Design review of the part built by this model. Coordinates are the model's own, in mm. Face numbers are marked on the shaded views. A direction names the side the tool comes from. Coordinates: 2 decimals unless noted, no trailing zeros. Loops run counter-clockwise (first coordinate to the right, second up) from the corner with the lowest first, then second, coordinate; pieces in that order, holes last. Notation, with made-up numbers: (-12.75, 80.5) -> (42.25, 80.5) arc R18 cw to (42.25, 100.5) -> close; hole circle Ø3 at (-31, 74.25). An arc over 180 degrees is marked (long way). Answer as a JSON object with one key per item and string values.
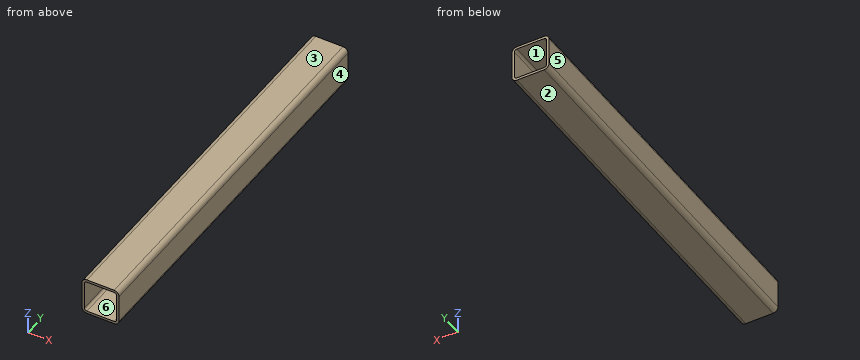
```python
from build123d import *

# Parameters (mm, degrees)
GB_T_6728_2002_SQUARE_HOLLOW_SECTION_60_DEPTH = 620


with BuildPart() as part:
    # Sketch1 → GB/T 6728-2002 square hollow section 60×60×4(1) (new body)
    with BuildSketch(Plane(origin=(0, 0, 0), x_dir=(-1, 0, 0), z_dir=(0, 1, 0))):
        with BuildLine():
            Line((-22, -30), (22, -30))
            ThreePointArc((22, -30), (27.656854249, -27.656854249), (30, -22))
            Line((30, -22), (30, 22))
            ThreePointArc((30, 22), (27.656854249, 27.656854249), (22, 30))
            Line((22, 30), (-22, 30))
            ThreePointArc((-22, 30), (-27.656854249, 27.656854249), (-30, 22))
            Line((-30, 22), (-30, -22))
            ThreePointArc((-30, -22), (-27.656854249, -27.656854249), (-22, -30))
        make_face()
        with BuildLine():
            Line((-22, -26), (22, -26))
            ThreePointArc((22, -26), (24.828427125, -24.828427125), (26, -22))
            Line((26, -22), (26, 22))
            ThreePointArc((26, 22), (24.828427125, 24.828427125), (22, 26))
            Line((22, 26), (-22, 26))
            ThreePointArc((-22, 26), (-24.828427125, 24.828427125), (-26, 22))
            Line((-26, 22), (-26, -22))
            ThreePointArc((-26, -22), (-24.828427125, -24.828427125), (-22, -26))
        make_face(mode=Mode.SUBTRACT)
    extrude(amount=GB_T_6728_2002_SQUARE_HOLLOW_SECTION_60_DEPTH)


solid = part.part
```
1) The part is to be moulded in two halves that separate along Z. For the marked faces 1, 2, 3 and 4, say which applies: pulls with the +Z half, pulls with the -Z half, needs draft (parallel to the pull), parting line crosses it, or undercut.
Completed:
{"face 1": "undercut", "face 2": "pulls with the -Z half", "face 3": "pulls with the +Z half", "face 4": "needs draft"}
2) Add section A-A, the plane y = 548.5. Give the boundary of the cut face in (x, z).
Completed:
{"outline": "(-30, -22) arc R8 ccw to (-22, -30) -> (22, -30) arc R8 ccw to (30, -22) -> (30, 22) arc R8 ccw to (22, 30) -> (-22, 30) arc R8 ccw to (-30, 22) -> close; hole (-26, -22) arc R4 ccw to (-22, -26) -> (22, -26) arc R4 ccw to (26, -22) -> (26, 22) arc R4 ccw to (22, 26) -> (-22, 26) arc R4 ccw to (-26, 22) -> close"}
3) For the marked faces 5 and 6, list the 3-axis set-ups (+Z, -Z, +X, -X, +Y, -Y) from which the entire face can be reached by the end or side of a thin tool; tool diameter is ignored.
Completed:
{"face 5": "+Z, -Z, -X, +Y, -Y", "face 6": "+Y, -Y"}
4) Add section C-C, the plane x = -11. Give the boundary of the cut face in (y, z), and give its area (3 significant figures).
Completed:
{"outline": "(0, -30) -> (620, -30) -> (620, -26) -> (0, -26) -> close; (0, 26) -> (620, 26) -> (620, 30) -> (0, 30) -> close", "area": "4,960 mm²"}
5) Add section B-B, the plane z = -7.5. Give the boundary of the cut face in (x, y).
Completed:
{"outline": "(-30, 0) -> (-26, 0) -> (-26, 620) -> (-30, 620) -> close; (26, 0) -> (30, 0) -> (30, 620) -> (26, 620) -> close"}
6) Wall thickness on probe 1 along X at (y, z) = (68.5, 2.5); probe 2 along X at (y, z) = (468, 24.5): over which ranges is each line inside the solid? List them lowest first.
Completed:
{"probe 1": "-30 to -26, 26 to 30", "probe 2": "-29.6 to -25.12, 25.12 to 29.6"}
